Here's how the part is built. I have some questions about the finished solid (model axes, mm). A direction names the side the tool comes from. Round coordinates to 2 decimals unless told otherwise and drop trailing zeros. Order: outer loops, then holes, each group sorted by start corner. A loop starts at its lowest first (then second) coordinate and runs counter-clockwise, first axis right, second up. Notation, with made-up numbers: M -11.75,-7 L 42.25,-7 A12 ccw 42.25,7 Z; hole C 18,4.25 d11. An arc over 180 degrees is marked long. Write each question's results on one line, items separated by ' | '. Start each with the question number.
```python
from build123d import *

# Parameters (mm, degrees)
SKETCH1_R           = 4
BOSS_EXTRUDE1_DEPTH = 36
CUT_EXTRUDE1_DEPTH  = 57
FILLET1_R           = 2
SKETCH3_R           = 7
CUT_EXTRUDE2_DEPTH  = 57


with BuildPart() as part:
    # Sketch1 → Boss-Extrude1 (new body)
    with BuildSketch(Plane.XY):
        with BuildLine():
            Line((0, 0), (0, -57.458281391))
            ThreePointArc((0, -57.458281391), (8.091910046, -67.274553225), (19.271838546, -61.204347325))
            Line((19.271838546, -61.204347325), (44, 0))
            Line((44, 0), (0, 0))
        make_face()
        with Locations((10, -57.458281391)):
            Circle(SKETCH1_R, mode=Mode.SUBTRACT)
    extrude(amount=-BOSS_EXTRUDE1_DEPTH)

    # Sketch2 → Cut-Extrude1 (cut)
    with BuildSketch(Plane.ZY):
        with BuildLine():
            Line((-32, -2), (-4, -2))
            ThreePointArc((-4, -2), (-3.292893219, -2.292893219), (-3, -3))
            Line((-3, -3), (-3, -57.458281391))
            Line((-3, -57.458281391), (-3, -71.28436633))
            Line((-3, -71.28436633), (-33, -71.28436633))
            Line((-33, -71.28436633), (-33, -57.458281391))
            Line((-33, -57.458281391), (-33, -3))
            ThreePointArc((-33, -3), (-32.707106781, -2.292893219), (-32, -2))
        make_face()
    extrude(amount=-CUT_EXTRUDE1_DEPTH, mode=Mode.SUBTRACT)

    # Fillet1
    fillet1_edges = [part.edges().sort_by_distance(p)[0] for p in [
        (22, 0, -36),
        (22, 0, 0),
    ]]
    fillet(fillet1_edges, radius=FILLET1_R)

    # Sketch3 → Cut-Extrude2 (cut)
    with BuildSketch(Plane(origin=(0, 0, 0), x_dir=(1, 0, 0), z_dir=(0, 1, 0))):
        with Locations(Location((20, 18, 0), (0, 0, 270))):
            Circle(SKETCH3_R)
    extrude(amount=-CUT_EXTRUDE2_DEPTH, mode=Mode.SUBTRACT)


solid = part.part
```
(1) I want a section at B-B on z = -18. Write out the boundary of the cut face in (x, y), and give its area (3 significant figures).
(2) I want a section at A-A on x = 10. Write out the boundary of the cut face in (y, z).
(3) I want a section at C-C on x = 20. Write out the boundary of the cut face in (y, z).
(4) On a 3-axis mill with a long thin cutter (end or side, diameter ignored), from which of +Z, -Z, +X, -X, +Y, -Y can I reach the whole of each face in a straight line? I mean faces 1 (the cylindrical face through (21.69, -0.6, -35.43)), 2 (the flat face through (16, -28, -3)). Say none if no direction works.
(5) If we mould it in two halves opening along Y, with no side actions, what happens to faces 3 (the cylindrical face through (9.479, -53.492, -1.479)), 4 (the cylindrical face through (7.903, -67.236, -1.479)), 5 (the cylindrical face through (15.741, -0.986, -23.555)), 6 (the flat face through (27.2, 0, -17.8))? For each: pulls with the +Y half, pulls with the -Y half, needs draft (parallel to the pull), parting line crosses it, or undercut.
(6) Please list where these lines run through material, in increasing order: line 1 (Z direction, x = 11, y = -30.5); line 2 (Y direction, x = 4, z = -22); line 3 (Y direction, x = 10, z = -34).
(7) I'm going to push flat-ended pins straight in: pin 1 Ø7 at (x, y) = (10, -57.46) entering from -Z; pin 2 Ø2 at (x, z) = (33, -20) entering from -Y; pin 3 Ø12 at (y, z) = (-21, -5) entering from +X. Where does each tip first touch, or does it pass through?
(8) I want a section at D-D on y = -19. Write out the boundary of the cut face in (x, z), and give its area (3 significant figures).
Solutions:
1) outline: M 0,-2 L 13,-2 L 13,0 L 0,0 Z; M 27,-2 L 43.19,-2 L 44,0 L 27,0 Z | area: 59.2 mm^2
2) outline: M -67.46,-36 L -61.46,-36 L -61.46,-33 L -67.46,-33 Z; M -67.46,-3 L -61.46,-3 L -61.46,0 L -67.46,0 Z; M -53.46,-36 L -2,-36 A2 ccw 0,-34 L 0,-2 A2 ccw -2,0 L -53.46,0 L -53.46,-3 L -3,-3 A1 cw -2,-4 L -2,-32 A1 cw -3,-33 L -53.46,-33 Z
3) outline: M -59.4,-36 L -2,-36 A2 ccw 0,-34 L 0,-25 L -2,-25 L -2,-32 A1 cw -3,-33 L -59.4,-33 Z; M -59.4,-3 L -3,-3 A1 cw -2,-4 L -2,-11 L 0,-11 L 0,-2 A2 ccw -2,0 L -59.4,0 Z
4) face 1: -Z, +X, -X, +Y | face 2: +X, -X, -Y
5) face 3: undercut | face 4: pulls with the -Y half | face 5: needs draft | face 6: pulls with the +Y half
6) line 1: -36 to -33, -3 to 0 | line 2: -2 to 0 | line 3: -67.46 to -61.46, -53.46 to 0
7) pin 1: through | pin 2: y = -2 | pin 3: x = 37.8
8) outline: M 0,-36 L 36.32,-36 L 36.32,-33 L 0,-33 Z; M 0,-3 L 36.32,-3 L 36.32,0 L 0,0 Z | area: 218 mm^2
